Read the model definition and answer for the solid it produces. Units are mm, in the model's axes. Coordinates: 2 decimals unless noted, no trailing zeros. Order: outer loops, then holes, each group sorted by start corner. A loop starts at its lowest first (then second) coordinate and runs counter-clockwise, first axis right, second up.
```python
from build123d import *

# Parameters (mm, degrees)
SKETCH_1_W          = 40
SKETCH_1_H          = 162
EXTRUDE_1_DEPTH     = 2
SKETCH_2_R          = 5.25
CUT_EXTRUDE_1_DEPTH = 3
SKETCH_4_W          = 30
SKETCH_4_H          = 10.5
SKETCH_4_W_2        = 29.434352085
SKETCH_4_H_2        = 10.438877802
CUT_EXTRUDE_4_DEPTH = 10
FILLET_2_R          = 2


with BuildPart() as part:
    # 草图1 → 凸台-拉伸1 (new body)
    with BuildSketch(Plane.XY):
        Rectangle(SKETCH_1_W, SKETCH_1_H)
    extrude(amount=EXTRUDE_1_DEPTH)

    # 草图2 → 切除-拉伸1 (cut)
    with BuildSketch(Plane.XY.offset(2)):
        with Locations((-10, 70)):
            Circle(SKETCH_2_R)
        with Locations((-10, -70)):
            Circle(SKETCH_2_R)
    extrude(amount=-CUT_EXTRUDE_1_DEPTH, mode=Mode.SUBTRACT)

    # 草图4 → 切除-拉伸4 (cut)
    with BuildSketch(Plane.XY.offset(2)):
        with Locations((5, 70)):
            Rectangle(SKETCH_4_W, SKETCH_4_H)
        with Locations((5.282823957, -70)):
            Rectangle(SKETCH_4_W_2, SKETCH_4_H_2)
    extrude(amount=-CUT_EXTRUDE_4_DEPTH, mode=Mode.SUBTRACT)

    # 圆角2
    fillet_2_edges = [part.edges().sort_by_distance(p)[0] for p in [
        (20, 75.25, 1),
        (20, 64.75, 1),
        (20, -64.780561099, 1),
        (20, -75.219438901, 1),
        (-20, 81, 1),
        (20, 81, 1),
        (20, -81, 1),
        (-20, -81, 1),
    ]]
    fillet(fillet_2_edges, radius=FILLET_2_R)


solid = part.part
```
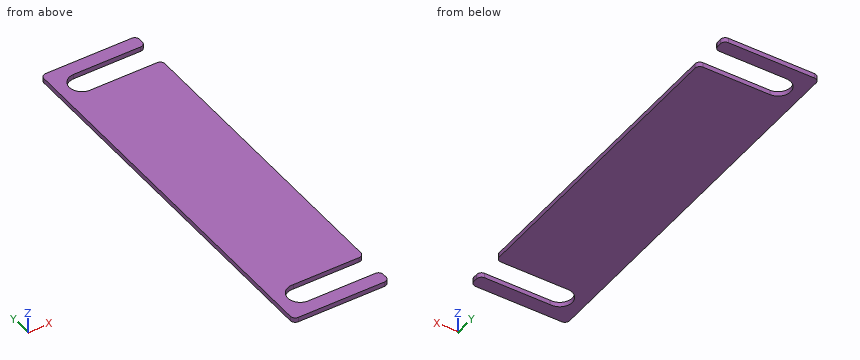
1) A cutting plane is placed at A-A, the plane x = 2.5. Determine the outline of the cut face in (y, z).
A:
outline: (-81, 0) - (-75.22, 0) - (-75.22, 2) - (-81, 2) - close; (-64.78, 0) - (64.75, 0) - (64.75, 2) - (-64.78, 2) - close; (75.25, 0) - (81, 0) - (81, 2) - (75.25, 2) - close
2) A cutting plane is placed at B-B, the plane z = 1.1. Determine the outline of the cut face in (x, y).
A:
outline: (-20, -79) arc R2 ccw to (-18, -81) - (18, -81) arc R2 ccw to (20, -79) - (20, -77.22) arc R2 ccw to (18, -75.22) - (-9.43, -75.22) arc R5.25 cw (long way) to (-9.43, -64.78) - (18, -64.78) arc R2 ccw to (20, -62.78) - (20, 62.75) arc R2 ccw to (18, 64.75) - (-10, 64.75) arc R5.25 cw to (-10, 75.25) - (18, 75.25) arc R2 ccw to (20, 77.25) - (20, 79) arc R2 ccw to (18, 81) - (-18, 81) arc R2 ccw to (-20, 79) - close
3) A flat-ended cylindrical pin translates along its axis: pin 1 Ø4 at (x, y) = (6.5, 25.5) entering from -Z. Find the tip coordinate at first contact, or state that the pin passes through.
A:
pin 1: stops at z = 0
4) Straight lines are drawn through the part: line 1 (Y direction, x = -9, z = 1.4); line 2 (X direction, y = -70, z = 0.95); line 3 (Y direction, x = -13, z = 1.25). For each, find the intervals that lie inside material, in ascending order.
A:
line 1: y = -81 to -75.22, -64.78 to 64.75, 75.25 to 81
line 2: x = -20 to -15.25
line 3: y = -81 to -74.31, -65.69 to 65.69, 74.31 to 81
5) A cutting plane is placed at C-C, the plane y = -70. Determine the outline of the cut face in (x, z).
A:
outline: (-20, 0) - (-15.25, 0) - (-15.25, 2) - (-20, 2) - close
